from build123d import *


with BuildPart() as part:
    # Sketch1 → Revolve1 (revolve)
    with BuildSketch(Plane(origin=(0, 0, 0), x_dir=(1, 0, 0), z_dir=(0, 1, 0))):
        Polygon((2.1, 0), (2.8, 0), (2.9, 0.1), (2.9, 1.1), (2.8, 1.2), (2.1, 1.2), (2, 1.1), (2, 0.1), align=None)
    revolve(axis=Axis((0, 0, 0), (0, 0, -1)))


solid = part.part
Could you check a few things on this model? Use its own coordinates, in mm. Give positions to 0.01 mm unless a question says otherwise; leave off trailing zeros. Order: outer loops, then holes, each group sorted by start corner. A loop starts at its lowest first (then second) coordinate and runs counter-clockwise, first axis right, second up.
1. Suppose I cut it at C-C (z = -0.3). Write out the boundary of the cut face in (x, y), plus the area to 3 significant figures.
Answers below:
outline: circle Ø5.8 at (0, 0); hole circle Ø4 at (0, 0)
area: 13.9 mm2
2. I need wall thicknesses on L1, parallel to Y at x = 0, z = -0.7; L2, parallel to Y at x = 2.1, z = -0.5. Which ranges of each line are inside material? Lowest first, please.
Answers below:
L1: y = -2.9 to -2, 2 to 2.9
L2: y = -2 to 2
3. Suppose I cut it at A-A (x = 0). Write out the boundary of the cut face in (y, z), plus the area to 3 significant figures.
Answers below:
outline: (-2.9, -1.1) - (-2.8, -1.2) - (-2.1, -1.2) - (-2, -1.1) - (-2, -0.1) - (-2.1, 0) - (-2.8, 0) - (-2.9, -0.1) - close; (2, -1.1) - (2.1, -1.2) - (2.8, -1.2) - (2.9, -1.1) - (2.9, -0.1) - (2.8, 0) - (2.1, 0) - (2, -0.1) - close
area: 2.12 mm2
4. Thinking about a two-plate mould opening in X: for faces 1 (the cylindrical face through (-0.434, 1.952, -0.593)), 2 (the cylindrical face through (-2.9, -0.1, -0.6)), which applies, +X half, -X half, draft (parallel to the pull), parting line (faces both ways), or undercut?
Answers below:
face 1: undercut
face 2: parting line
